Here's the drawing with two shaded views (mm, measured from the low corner). I have some questions. Round coordinates to 2 decimals unless told otherwise and drop trailing zeros. Loops run counter-clockwise (first coordinate to the right, second up) from the corner with the lowest first, then second, coordinate; pieces in that order, holes last.
(1) If I drill on line 1 along X through (y, z) = (0.95, 1.3); line 2 along Y through (x, z) = (12, 0.2); line 3 along Z through (x, y) = (10.25, 1.05), over which ranges is the centre line in solid material (lowest first)?
(2) I want a section at D-D on x = 6.25. Write out the boundary of the cut face in (y, z), plus the area to 3 significant figures.
(3) Will these pins go through, and if not, where does the flat tip stop? pin 1 Ø0.6 at (y, z) = (1, 1.5) entering from +X; pin 2 Ø0.6 at (x, z) = (12, 1.5) entering from -Y.
(4) I want a section at B-B on x = 12. Write out the boundary of the cut face in (y, z).
(5) I want a section at A-A on z = 0.75. Write out the boundary of the cut face in (x, y), plus the area to 3 significant figures.
(6) I want a section at C-C on y = 1. Write out the boundary of the cut face in (x, z), plus the area to 3 significant figures.
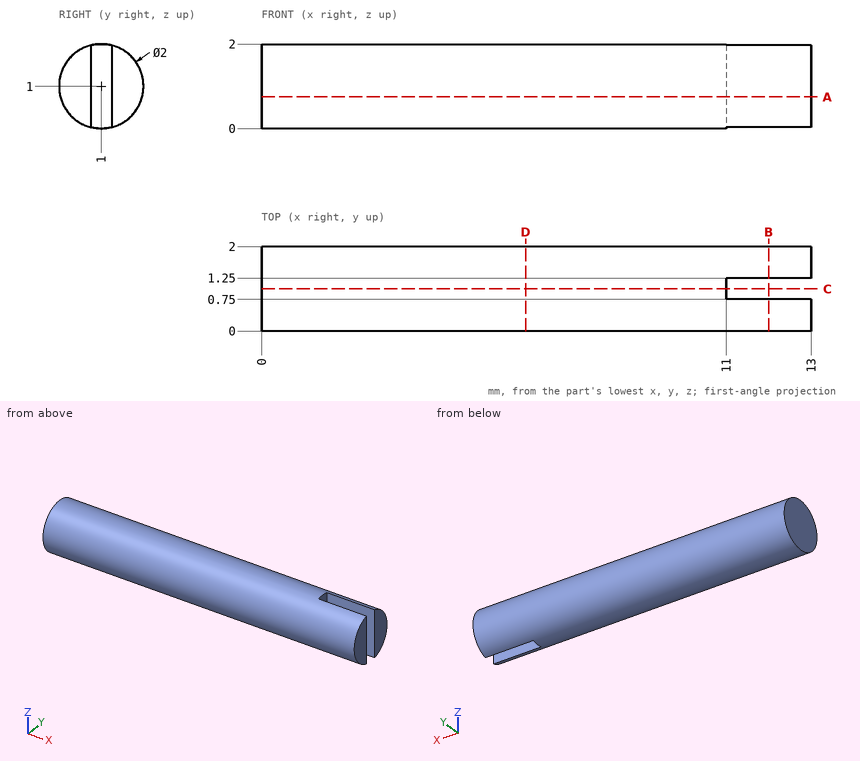
Filled sheet:
1. line 1: x = 0 to 11
1. line 2: y = 0.4 to 0.75, 1.25 to 1.6
1. line 3: z = 0 to 2
2. outline: circle Ø2 at (1, 1)
2. area: 3.14 mm2
3. pin 1: stops at x = 13
3. pin 2: stops at y = 0.02
4. outline: (0.75, 0.03) - (0.75, 1.97) arc R1 ccw to start; (1.25, 0.03) arc R1 ccw to (1.25, 1.97) - close
5. outline: (0, 0.03) - (13, 0.03) - (13, 0.75) - (11, 0.75) - (11, 1.25) - (13, 1.25) - (13, 1.97) - (0, 1.97) - close
5. area: 24.2 mm2
6. outline: (0, 0) - (11, 0) - (11, 2) - (0, 2) - close
6. area: 22.0 mm2
